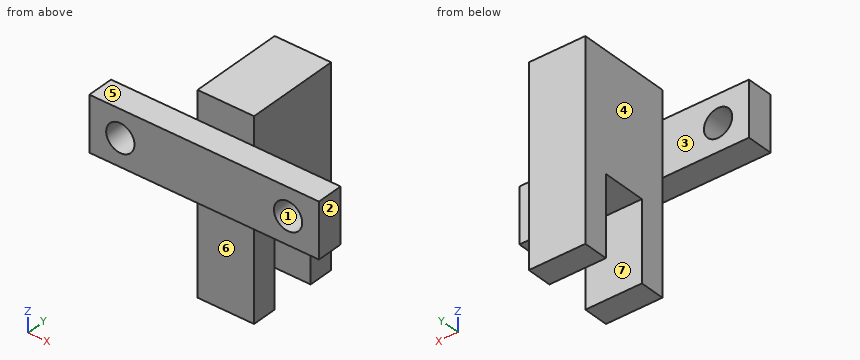
```python
from build123d import *

# Parameters (mm, degrees)
SKETCH_1_W          = 26
SKETCH_1_H          = 6.2
EXTRUDE_1_DEPTH     = 3
SKETCH_2_W          = 6.4
SKETCH_2_H          = 22.2
EXTRUDE_2_DEPTH     = 10.7
SKETCH_3_W          = 9
SKETCH_3_H          = 5
CUT_EXTRUDE_1_DEPTH = 10.7
SKETCH_4_R          = 1.6
CUT_EXTRUDE_2_DEPTH = 10.7


with BuildPart() as part:
    # 草图1 → 凸台-拉伸1 (new body)
    with BuildSketch(Plane(origin=(0, 0, 0), x_dir=(1, 0, 0), z_dir=(0, 1, 0))):
        Rectangle(SKETCH_1_W, SKETCH_1_H)
    extrude(amount=EXTRUDE_1_DEPTH)

    # 草图2 → 凸台-拉伸2 (add)
    with BuildSketch(Plane(origin=(0, 3, 0), x_dir=(1, 0, 0), z_dir=(0, 1, 0))):
        with Locations((0, 4.8)):
            Rectangle(SKETCH_2_W, SKETCH_2_H)
    extrude(amount=EXTRUDE_2_DEPTH)

    # 草图3 → 切除-拉伸1 (cut)
    with BuildSketch(Plane.ZY.offset(3.2)):
        with Locations((-11.4, 8.35)):
            Rectangle(SKETCH_3_W, SKETCH_3_H)
    extrude(amount=-CUT_EXTRUDE_1_DEPTH, mode=Mode.SUBTRACT)

    # 草图4 → 切除-拉伸2 (cut)
    with BuildSketch(Plane(origin=(0, 3, 0), x_dir=(1, 0, 0), z_dir=(0, 1, 0))):
        with Locations(Location((-9.5, 0, 0), (0, 0, 270))):
            Circle(SKETCH_4_R)
        with Locations(Location((9.5, 0, 0), (0, 0, 270))):
            Circle(SKETCH_4_R)
    extrude(amount=-CUT_EXTRUDE_2_DEPTH, mode=Mode.SUBTRACT)


solid = part.part
```
Part model, mm, in its own coordinate system. Face numbers are marked on the shaded views. A direction names the side the tool comes from. Round coordinates to 2 decimals unless told otherwise and drop trailing zeros. Loops run counter-clockwise (first coordinate to the right, second up) from the corner with the lowest first, then second, coordinate; pieces in that order, holes last.
Item 1: Drop flat-ended pins along their axis: P1, Ø3, axis at x = 0, z = -9, coming from the -Y side; P2, Ø4, axis at y = 10.5, z = -5.5, coming from the -X side; P3, Ø5, axis at x = 7, z = -11, coming from the +Y side; P4, Ø6, axis at y = 5.5, z = -12.5, coming from the +X side. Give the stop position or say it passes through.
Item 2: 3-axis set-ups, long thin cutter, end or side, ignore diameter. For the marked faces 4, 5, 6 and 7: which of +Z, -Z, +X, -X, +Y, -Y reach the whole face in a straight line?
Item 3: Cut at A-A, the plane z = 0. Give the cut face in (x, y).
Item 4: Cut at B-B, the plane x = 9.5. Give the cut face in (y, z).
Item 5: Mould opens along X. For the marked faces 1, 2 and 3 say: +X half, -X half, draft (parallel to the pull), parting line (faces both ways), or undercut.
Item 6: Cut at D-D, the plane y = 4.5. Give the cut face in (x, z), then the cut area to 3 significant figures.
Item 7: Cut at C-C, the plane z = -2.75. Give the cut face in (x, y).
Item 8: Drill centre lines: line 1 (X direction, y = 1.1, z = 0); line 2 (Y direction, x = 2, z = 3.75); line 3 (X direction, y = 10.25, z = -1.5). Where is each one in solid material? Low to high.
A:
1. P1: stops at y = 3
1. P2: stops at x = -3.2
1. P3: passes through
1. P4: stops at x = 3.2
2. face 4: +Z, -Z, -X, +Y
2. face 5: +Z, +X, -X, -Y
2. face 6: -Z, +X, -X, -Y
2. face 7: -Z, +X, -X
3. outline: (-13, 0) - (-11.1, 0) - (-11.1, 3) - (-13, 3) - close; (-7.9, 0) - (7.9, 0) - (7.9, 3) - (3.2, 3) - (3.2, 13.7) - (-3.2, 13.7) - (-3.2, 3) - (-7.9, 3) - close; (11.1, 0) - (13, 0) - (13, 3) - (11.1, 3) - close
4. outline: (0, -3.1) - (3, -3.1) - (3, -1.6) - (0, -1.6) - close; (0, 1.6) - (3, 1.6) - (3, 3.1) - (0, 3.1) - close
5. face 1: undercut
5. face 2: +X half
5. face 3: draft
6. outline: (-3.2, -15.9) - (3.2, -15.9) - (3.2, 6.3) - (-3.2, 6.3) - close
6. area: 142 mm2
7. outline: (-13, 0) - (13, 0) - (13, 3) - (3.2, 3) - (3.2, 13.7) - (-3.2, 13.7) - (-3.2, 3) - (-13, 3) - close
8. line 1: x = -13 to -11.1, -7.9 to 7.9, 11.1 to 13
8. line 2: y = 3 to 13.7
8. line 3: x = -3.2 to 3.2
